from build123d import *

# Parameters (mm, degrees)
SKETCH_1_R               = 80
SKETCH_1_R_2             = 40.5
EXTRUDE_1_DEPTH          = 5
SKETCH_3_R               = 1.5
SKETCH_5_R               = 1.5
CUT_EXTRUDE_2_DEPTH      = 55
PATTERN_CIRCULAR_1_COUNT = 3


with BuildPart() as part:
    # 草图1 → 凸台-拉伸1 (new body)
    with BuildSketch(Plane.XY):
        Circle(SKETCH_1_R)
        Circle(SKETCH_1_R_2, mode=Mode.SUBTRACT)
    extrude(amount=EXTRUDE_1_DEPTH)

    # 切除-扫描1: sweep along a path in 草图2
    with BuildLine(Plane.XY.offset(5)) as sweep_1_path:
        CenterArc((0, 0), 55, 0, 360)
    # 草图3 → 切除-扫描1 (sweep, cut)
    with BuildSketch(Plane(origin=(0, 0, 0), x_dir=(0, 0, -1), z_dir=(1, 0, 0))):
        with Locations((-5, 55)):
            Circle(SKETCH_3_R)
    sweep(path=sweep_1_path.line, mode=Mode.SUBTRACT)

    # 草图5 → 切除-拉伸2 (cut)
    with BuildSketch(Plane(origin=(0, 0, 0), x_dir=(1, 0, 0), z_dir=(0, 1, 0))):
        with Locations((0, -5)):
            Circle(SKETCH_5_R)
    cut_extrude_2 = extrude(amount=CUT_EXTRUDE_2_DEPTH, mode=Mode.SUBTRACT)

    # 阵列(圆周)1: 切除-拉伸2 ×3 about axis
    pattern_circular_1_axis = Axis((0, 0, 5), (0, 0, -1))
    for i in range(1, PATTERN_CIRCULAR_1_COUNT):
        add(cut_extrude_2.rotate(pattern_circular_1_axis, i * 360 / PATTERN_CIRCULAR_1_COUNT), mode=Mode.SUBTRACT)


solid = part.part
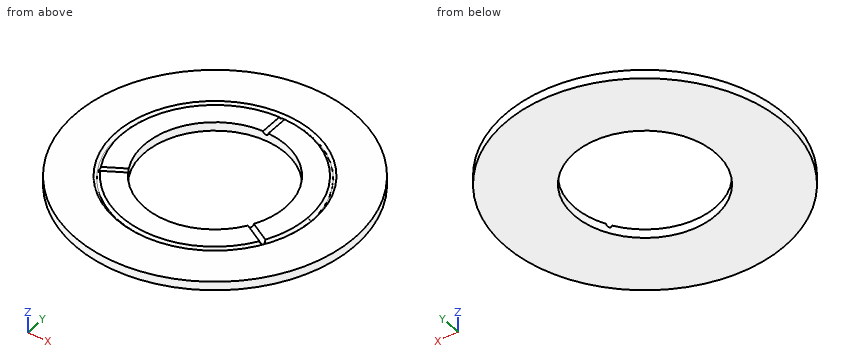
Input: part model. Units: mm. Frame: model coordinates. Give positions to 0.01 mm unless a question says otherwise; leave off trailing zeros. Loops run counter-clockwise (first coordinate to the right, second up) from the corner with the lowest first, then second, coordinate; pieces in that order, holes last. Notation, with made-up numbers: (19.25, 30) -> (78.25, 30) arc R22 ccw to (78.25, 59) -> close; hole circle Ø5 at (-19.75, 14). An arc over 180 degrees is marked (long way). Answer as a JSON object with one key per item and string values. Group by question number.
Item 1: Pin query (flat end, axial travel): P1, Ø1, axis at y = -27.5, z = 3.5, coming from the +X side; P2, Ø3, axis at y = 43, z = 4, coming from the +X side; P3, Ø10, axis at x = -42.5, y = -3.5, coming from the -Z side. Return the tip coordinate at first contact, or that it passes through.
Item 2: Line query: probe 1 along Y at (x, z) = (0, 3.15); probe 2 along X at (y, z) = (1, 1.3); probe 3 along X at (y, z) = (31, 4.15). Output: solid intervals per line, ascending.
Item 3: Cut plane A-A, the plane z = 2.15. Return the cut outline in (x, y), and give its area (3 significant figures).
Checks:
{
 "1": {"P1": "stops at x = 75.31", "P2": "stops at x = 68.39", "P3": "stops at z = 0"},
 "2": {"probe 1": "y = -80 to -40.5, 40.5 to 80", "probe 2": "x = -79.99 to -40.49, 40.49 to 79.99", "probe 3": "x = -73.75 to -46.92, -43.93 to -26.06, 26.06 to 43.93, 46.92 to 73.75"},
 "3": {"outline": "circle Ø160 at (0, 0); hole circle Ø81 at (0, 0)", "area": "15,000 mm²"}
}
